Geometry check sheet. Reference: drawing and pictorial views, mm from the part's lowest x, y, z. A direction names the side the tool comes from. Give positions to 0.01 mm unless a question says otherwise; leave off trailing zeros. Order: outer loops, then holes, each group sorted by start corner. A loop starts at its lowest first (then second) coordinate and runs counter-clockwise, first axis right, second up. Notation, with made-up numbers: (47.5, -1.5) -> (51.5, -1.5) arc R23 cw to (51.5, 8.5) -> close; hole circle Ø1 at (22, 21.25). An arc over 180 degrees is marked (long way). Write each question's results on one line, items separated by ' | '. Start each with the question number.
1. Cross-section at D-D, the plane z = 5.5. Enter the section's corners in (x, y).
2. Depth check by flat-ended pin: pin 1 Ø1 at (x, z) = (14.5, 42) entering from +Y; pin 2 Ø3 at (x, z) = (7.5, 31) entering from -Y. Enter the tip coordinate at first touch or a pass-through.
3. Cross-section at A-A, the plane x = 10. Enter the section's corners in (y, z).
4. Set-up check for the marked faces 1, 2 and 3: record each of +Z, -Z, +X, -X, +Y, -Y from which the full face is reachable in a straight line by a thin tool's end or side.
5. Material ranges on L1, parallel to Z at x = 16.75, y = 15.75; L2, parallel to Y at x = 10.25, z = 36.5; L3, parallel to X at y = 14, z = 47.5, recorded low to high. Write a range as from..to.
6. Cross-section at C-C, the plane z = 29. Enter the section's corners in (x, y), then the cut area to 3 significant figures.
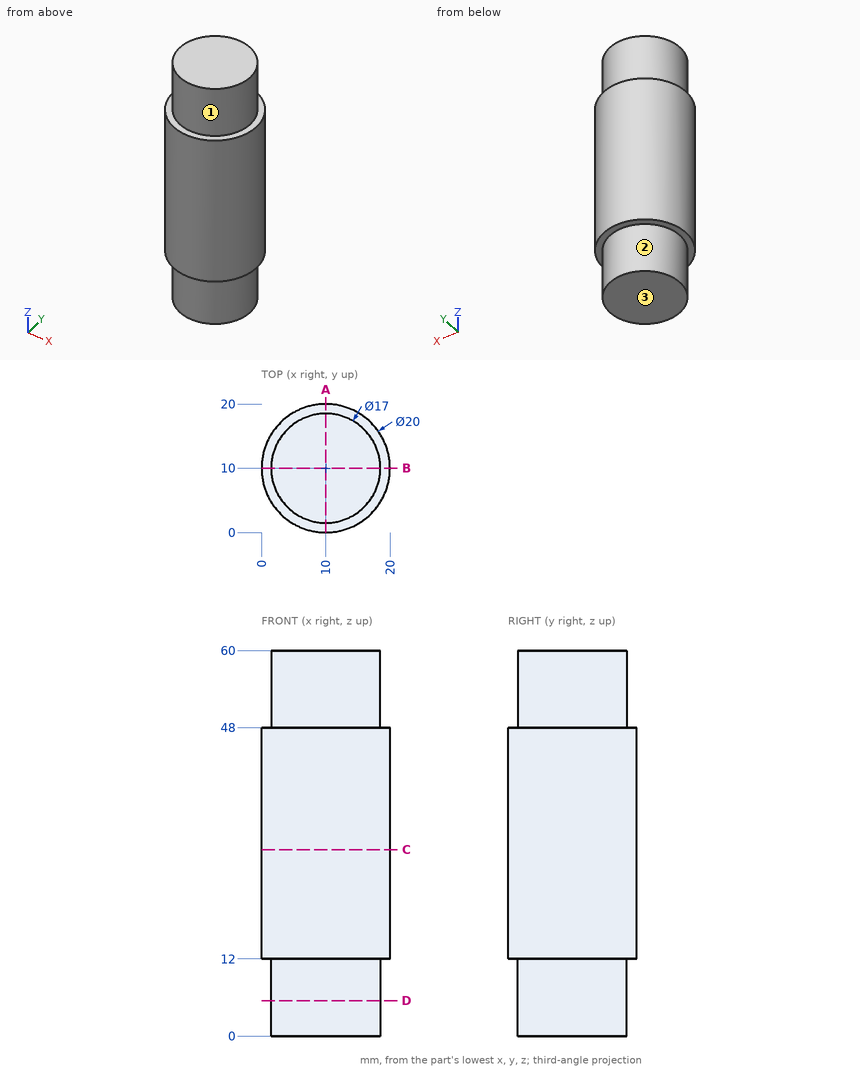
Results below:
1) outline: circle Ø17 at (10, 10)
2) pin 1: stops at y = 19.17 | pin 2: stops at y = 0.05
3) outline: (0, 12) -> (1.5, 12) -> (1.5, 0) -> (18.5, 0) -> (18.5, 12) -> (20, 12) -> (20, 48) -> (18.5, 48) -> (18.5, 60) -> (1.5, 60) -> (1.5, 48) -> (0, 48) -> close
4) face 1: +Z | face 2: -Z | face 3: -Z, +X, -X, +Y, -Y
5) L1: z = 12..48 | L2: y = 0..20 | L3: x = 0.83..19.17
6) outline: circle Ø20 at (10, 10) | area: 314 mm²
